from build123d import *

# Parameters (mm, degrees)
SKETCH_1_R                   = 7.5
EXTRUDE_1_DEPTH              = 207
SKETCH_2_R                   = 10
EXTRUDE_2_DEPTH              = 43
SKETCH_3_OUTSIDE_W           = 72.318
SKETCH_3_OUTSIDE_H           = 72.318
SKETCH_3_OUTSIDE_W_2         = 23
SKETCH_3_OUTSIDE_H_2         = 18
CUT_EXTRUDE_1_DEPTH          = 20
HOLE_WIZARD_M8_1_D           = 6.8
HOLE_WIZARD_M8_1_DEPTH       = 18.25
HOLE_WIZARD_M8_1_CSINK_D     = 8.05
HOLE_WIZARD_M8_1_CSINK_ANGLE = 90
HOLE_WIZARD_M8_1_TIP         = 2.042926105


with BuildPart() as part:
    # 草图1 → 凸台-拉伸1 (new body)
    with BuildSketch(Plane.XY):
        Circle(SKETCH_1_R)
    extrude(amount=EXTRUDE_1_DEPTH)

    # 草图2 → 凸台-拉伸2 (add)
    with BuildSketch(Plane(origin=(0, 0, 0), x_dir=(-1, 0, 0), z_dir=(0, 0, -1))):
        Circle(SKETCH_2_R)
    extrude(amount=EXTRUDE_2_DEPTH)

    # 草图3 outside → 切除-拉伸1 (cut)
    with BuildSketch(Plane(origin=(0, 0, -43), x_dir=(-1, 0, 0), z_dir=(0, 0, -1))):
        Rectangle(SKETCH_3_OUTSIDE_W, SKETCH_3_OUTSIDE_H)
        Rectangle(SKETCH_3_OUTSIDE_W_2, SKETCH_3_OUTSIDE_H_2, mode=Mode.SUBTRACT)
    extrude(amount=-CUT_EXTRUDE_1_DEPTH, mode=Mode.SUBTRACT)

    # M8 螺纹孔1
    with Locations(Plane(origin=(0, 0, -43), x_dir=(-1, 0, 0), z_dir=(0, 0, -1))):
        with Locations((0, 0)):
            CounterSinkHole(HOLE_WIZARD_M8_1_D / 2, HOLE_WIZARD_M8_1_CSINK_D / 2, depth=HOLE_WIZARD_M8_1_DEPTH, counter_sink_angle=HOLE_WIZARD_M8_1_CSINK_ANGLE)
            with Locations((0, 0, -(HOLE_WIZARD_M8_1_DEPTH + HOLE_WIZARD_M8_1_TIP / 2))):  # 118° drill point
                Cone(0, HOLE_WIZARD_M8_1_D / 2, HOLE_WIZARD_M8_1_TIP, mode=Mode.SUBTRACT)


solid = part.part
Check sheet for the modelled part. Datum: model origin and axes. Units: mm. A direction names the side the tool comes from. Round coordinates to 2 decimals unless told otherwise and drop trailing zeros. Loops run counter-clockwise (first coordinate to the right, second up) from the corner with the lowest first, then second, coordinate; pieces in that order, holes last. Notation, with made-up numbers: (75.5, -2) - (127.5, -2) arc R14 ccw to (127.5, 17) - close; hole circle Ø10 at (4.25, 80). An arc over 180 degrees is marked (long way). Answer as CSV lines item,"result". Start each with the question number.
Item 1: Release check for a two-part mould opening along Y. For faces 4 (the cylindrical face through (-0.74, -3.32, -33.44)), 5 (the cylindrical face through (-7.493, 0.33, 102.051)), 6 (the flat face through (0, -9, -33)) record: +Y half, -Y half, draft (parallel to the pull), parting line (faces both ways), or undercut.
Item 2: Section check A-A (z = 8). Record the boundary of the cut face in (x, y), and give its area (3 significant figures).
Item 3: Scan lines: line 1 (Y direction, x = 0, z = -36.25); line 2 (X direction, y = 0, z = -34.5); line 3 (X direction, y = 0.25, z = 179). Record each from-to range of solid material in increasing order. Write a range as [from, to].
Item 4: Depth check by flat-ended pin: P1, Ø12, axis at y = -3.5, z = -7, coming from the +X side; P2, Ø8, axis at y = -3, z = 124.5, coming from the +X side; P3, Ø5, axis at x = -7.5, y = 7, coming from the +Z side; P4, Ø10, axis at y = 3, z = 61, coming from the -X side. Enter the tip coordinate at first touch or a pass-through.
Item 5: Set-up check for faces 1 (the flat face through (0, 9, -33)), 2 (the flat face through (0, 0, 207)), 3 (the flat face through (-4, 7, 0)): record each of +Z, -Z, +X, -X, +Y, -Y from which the full face is reachable in a straight line by a thin tool's end or side.
Report:
1,face 4,"undercut"
1,face 5,"parting line"
1,face 6,"-Y half"
2,outline,"circle Ø15 at (0, 0)"
2,area,"177 mm2"
3,line 1,"y = [-9, -3.4], [3.4, 9]"
3,line 2,"x = [-10, -3.4], [3.4, 10]"
3,line 3,"x = [-7.5, 7.5]"
4,P1,"stops at x = 10"
4,P2,"stops at x = 7.5"
4,P3,"stops at z = 0"
4,P4,"stops at x = -7.5"
5,face 1,"-Z, +X, -X, +Y"
5,face 2,"+Z, +X, -X, +Y, -Y"
5,face 3,"+Z"
